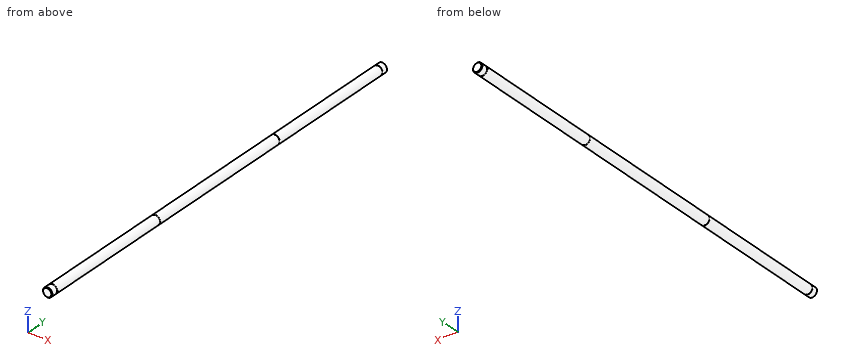
```python
from build123d import *

# Parameters (mm, degrees)
SKETCH1_R           = 7.5
BOSS_EXTRUDE1_DEPTH = 688
SKETCH2_R           = 7.5
SKETCH2_R_2         = 7.15
CUT_EXTRUDE1_DEPTH  = 1.1
CHAMFER1_SIZE       = 1
SKETCH3_R           = 7.5
SKETCH3_R_2         = 7.15
CUT_EXTRUDE2_DEPTH  = 1.1


with BuildPart() as part:
    # Sketch1 → Boss-Extrude1 (new body)
    with BuildSketch(Plane(origin=(0, 0, 0), x_dir=(1, 0, 0), z_dir=(0, 1, 0))):
        with Locations(Location((0, 0, 0), (0, 0, 270))):
            Circle(SKETCH1_R)
    extrude(amount=BOSS_EXTRUDE1_DEPTH)

    # Sketch2 → Cut-Extrude1 (cut)
    with BuildSketch(Plane(origin=(0, 10, 0), x_dir=(-1, 0, 0), z_dir=(0, -1, 0))):
        with Locations(Location((0, 0, 0), (0, 0, 90))):
            Circle(SKETCH2_R)
        with Locations(Location((0, 0, 0), (0, 0, 90))):
            Circle(SKETCH2_R_2, mode=Mode.SUBTRACT)
    cut_extrude1 = extrude(amount=-CUT_EXTRUDE1_DEPTH, mode=Mode.SUBTRACT)

    # Chamfer1
    chamfer1_edges = [part.edges().sort_by_distance(p)[0] for p in [
        (0, 0, -7.5),
        (0, 688, -7.5),
    ]]
    chamfer(chamfer1_edges, length=CHAMFER1_SIZE)

    # Sketch3 → Cut-Extrude2 (cut)
    with BuildSketch(Plane(origin=(0, 221, 0), x_dir=(-1, 0, 0), z_dir=(0, -1, 0))):
        with Locations(Location((0, 0, 0), (0, 0, 90))):
            Circle(SKETCH3_R)
        with Locations(Location((0, 0, 0), (0, 0, 90))):
            Circle(SKETCH3_R_2, mode=Mode.SUBTRACT)
    cut_extrude2 = extrude(amount=-CUT_EXTRUDE2_DEPTH, mode=Mode.SUBTRACT)

    # Mirror1: Cut-Extrude1, Cut-Extrude2 across plane
    add(cut_extrude1.mirror(Plane(origin=(0, 344, 0), x_dir=(0, 0, 1), z_dir=(0, -1, 0))), mode=Mode.SUBTRACT)
    add(cut_extrude2.mirror(Plane(origin=(0, 344, 0), x_dir=(0, 0, 1), z_dir=(0, -1, 0))), mode=Mode.SUBTRACT)


solid = part.part
```
Geometry: final body of the model. Coordinates: model frame, mm. Give positions to 0.01 mm unless a question says otherwise; leave off trailing zeros. Order: outer loops, then holes, each group sorted by start corner. A loop starts at its lowest first (then second) coordinate and runs counter-clockwise, first axis right, second up. Notation, with made-up numbers: M 67.25,19 L 108.25,19 A20 cw 108.25,36 Z; hole C 23.25,-20 d5. An arc over 180 degrees is marked long. Answer as CSV lines item,"result". Start each with the question number.
1) First-contact query: P1, Ø6, axis at x = -3.5, y = 492, coming from the +Z side; P2, Ø7.5, axis at x = 0.5, z = 1, coming from the -Y side; P3, Ø3, axis at y = 549, z = -2.5, coming from the -X side; P4, Ø2, axis at y = 155.5, z = 4, coming from the -X side. Flat tips, straight axial feed; report the tip coordinate or a pass-through.
2) Line query: line 1 (Z direction, x = 3.75, y = 129.5); line 2 (Z direction, x = 3.5, y = 104); line 3 (X direction, y = 251, z = -0.75). Output: solid intervals per line, ascending. Write a range as from..to.
3) Cut plane A-A (y = 448). Output: boundary loops of the cut face in (x, z).
Findings below:
1,P1,"stops at z = 7.48"
1,P2,"stops at y = 0"
1,P3,"stops at x = -7.43"
1,P4,"stops at x = -6.87"
2,line 1,"z = -6.5..6.5"
2,line 2,"z = -6.63..6.63"
2,line 3,"x = -7.46..7.46"
3,outline,"C 0,0 d15"
